Verification items for the finished model (mm, model axes). Face numbers are marked on the shaded views. Give positions to 0.01 mm unless a question says otherwise; leave off trailing zeros. Loops run counter-clockwise (first coordinate to the right, second up) from the corner with the lowest first, then second, coordinate; pieces in that order, holes last. Notation, with made-up numbers: (81, -28) - (92, -28) arc R25 ccw to (92, 11) - close; hole circle Ø4 at (50.25, 19.25). An arc over 180 degrees is marked (long way). Answer in a Markdown table with one row per item.
```python
from build123d import *
from OCP.BRepFilletAPI import BRepFilletAPI_MakeChamfer

# Parameters (mm, degrees)
SKETCH_1_W          = 87
SKETCH_1_H          = 44
EXTRUDE_1_DEPTH     = 6
SKETCH_2_R          = 8.179245246
CUT_EXTRUDE_1_DEPTH = 6
CHAMFER_1_SIZE      = 8.5
CHAMFER_1_SIZE2     = 9.987134599


with BuildPart() as part:
    # 草图1 → 凸台-拉伸1 (new body)
    with BuildSketch(Plane.XY):
        Rectangle(SKETCH_1_W, SKETCH_1_H)
    extrude(amount=EXTRUDE_1_DEPTH)

    # 草图2 → 切除-拉伸1 (cut)
    with BuildSketch(Plane.XY.offset(6)):
        Circle(SKETCH_2_R)
        Polygon((-43.5, -22), (-37.316203273, 22), (-43.5, 22), align=None)
        Polygon((43.5, -22), (37.316203273, 22), (43.5, 22), align=None)
    extrude(amount=-CUT_EXTRUDE_1_DEPTH, mode=Mode.SUBTRACT)

    # 倒角1: one chamfer whose edges measure the first distance from different faces: ONE call of the kernel's chamfer builder (chamfer() names one face for all edges)
    chamfer_1_edges_1 = [part.edges().sort_by_distance(p)[0] for p in [
        (37.316203273, 22, 3),
    ]]
    chamfer_1_side_1 = [part.faces().sort_by_distance(p)[0] for p in [
        (0, 22, 3),
    ]]
    chamfer_1_edges_2 = [part.edges().sort_by_distance(p)[0] for p in [
        (-37.316203273, 22, 3),
    ]]
    chamfer_1_side_2 = [part.faces().sort_by_distance(p)[0] for p in [
        (-40.408101637, 0, 3),
    ]]
    chamfer_1 = BRepFilletAPI_MakeChamfer(part.part.solid().wrapped)
    for e in chamfer_1_edges_1:
        chamfer_1.Add(CHAMFER_1_SIZE, CHAMFER_1_SIZE2, e.wrapped, chamfer_1_side_1[0].wrapped)  # the first distance lies on this face
    for e in chamfer_1_edges_2:
        chamfer_1.Add(CHAMFER_1_SIZE, CHAMFER_1_SIZE2, e.wrapped, chamfer_1_side_2[0].wrapped)  # the first distance lies on this face
    add(Compound.cast(chamfer_1.Shape()), mode=Mode.REPLACE)


solid = part.part
```
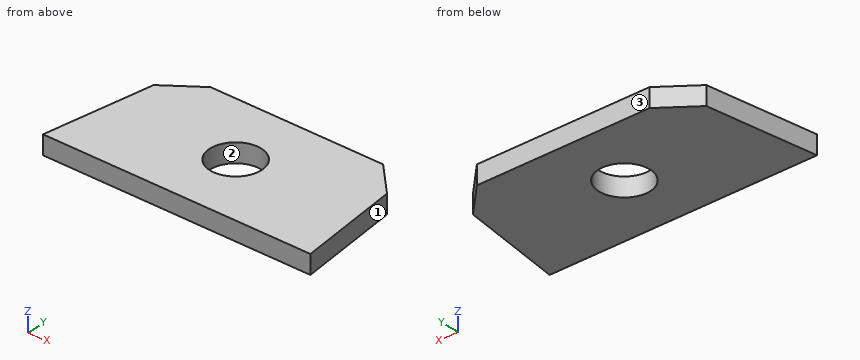
Q1. Sectioned sample at D-D (y = -13). Record the cut outline in (x, z).
Completed:
| item | result |
|---|---|
| outline | (-42.24, 0) - (42.24, 0) - (42.24, 6) - (-42.24, 6) - close |
Q2. Go/stop test with a flat-tipped pin: P1, Ø1.5, axis at x = -30, z = 4.5, coming from the +Y side. Record where the tip stops, or that it passes through.
Completed:
| item | result |
|---|---|
| P1 | y = 20.55 |
Q3. Thickness scan on line 1 (Y direction, x = 0, z = 3.85); line 2 (X direction, y = 5, z = 0.55); line 3 (X direction, y = 3, z = 0.7). Record the ranges inside material, lowest first.
Completed:
| item | result |
|---|---|
| line 1 | -22 to -8.18, 8.18 to 22 |
| line 2 | -39.71 to -6.47, 6.47 to 39.71 |
| line 3 | -39.99 to -7.61, 7.61 to 39.99 |
Q4. Sectioned sample at A-A (x = 0). Record the cut outline in (y, z), and give its area (3 significant figures).
Completed:
| item | result |
|---|---|
| outline | (-22, 0) - (-8.18, 0) - (-8.18, 6) - (-22, 6) - close; (8.18, 0) - (22, 0) - (22, 6) - (8.18, 6) - close |
| area | 166 mm^2 |
Q5. Draft check along X on the marked faces 1, 2 and 3. Enter one of: +X half, -X half, draft (parallel to the pull), parting line (faces both ways), or undercut.
Completed:
| item | result |
|---|---|
| face 1 | +X half |
| face 2 | undercut |
| face 3 | draft |
Q6. Sectioned sample at C-C (y = -6). Record the cut outline in (x, z), and give its area (3 significant figures).
Completed:
| item | result |
|---|---|
| outline | (-41.25, 0) - (-5.56, 0) - (-5.56, 6) - (-41.25, 6) - close; (5.56, 0) - (41.25, 0) - (41.25, 6) - (5.56, 6) - close |
| area | 428 mm^2 |
Q7. Sectioned sample at B-B (z = 3.6). Record the cut outline in (x, y), and give its area (3 significant figures).
Completed:
| item | result |
|---|---|
| outline | (-43.5, -22) - (43.5, -22) - (38.71, 12.11) - (28.82, 22) - (-27.33, 22) - (-38.5, 13.58) - close; hole circle Ø16.36 at (0, 0) |
| area | 3,260 mm^2 |
